```python
from build123d import *


with BuildPart() as part:
    # Sweep1: sweep along a path in Sketch1
    with BuildLine(Plane.XY) as sweep1_path:
        Line((0, 8), (1060, 8))
        ThreePointArc((1060, 8), (1068, 0), (1060, -8))
        Line((1060, -8), (0, -8))
        ThreePointArc((0, -8), (-8, 0), (0, 8))
    # Sketch2 → Sweep1 (sweep)
    with BuildSketch(Plane(origin=(0, 0, 0), x_dir=(0, 0, -1), z_dir=(1, 0, 0))):
        with BuildLine():
            Line((-10, 8), (10, 8))
            ThreePointArc((10, 8), (0, 18), (-10, 8))
        make_face()
    sweep(path=sweep1_path.line)


solid = part.part
```
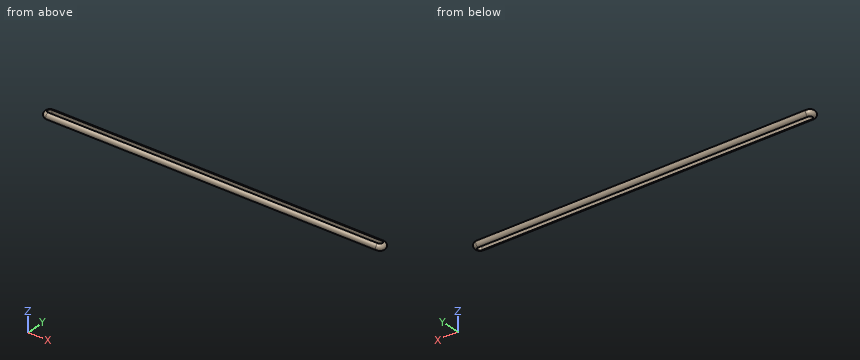
Verification items for the finished model (mm, model axes). Coordinates: 2 decimals unless noted, no trailing zeros. Write each loop counter-clockwise with the first axis right and the second up, starting at its lowest first coordinate (ties: lowest second). Pieces come first, ordered by that corner, then holes. Notation, with made-up numbers: (18.25, 76) - (68.25, 76) arc R8 ccw to (68.25, 82) - close; hole circle Ø10 at (45.5, 45.5). An arc over 180 degrees is marked (long way). One line per question, with ' | ' between items. Start each with the question number.
1. Section check A-A (x = 734). Enter the section's corners in (y, z).
2. Gauge pin test, flat ends, axial feed: P1, Ø4, axis at x = 254, y = -5.5, coming from the +Z side; P2, Ø3, axis at x = 107, y = -11, coming from the -Z side; P3, Ø4, axis at x = 477, z = -3.5, coming from the +Y side. Record the tip position at first contact, or that the pin passes through.
3. Material ranges on line 1 along Y through (x, z) = (796, 0.5); line 2 along Y through (x, z) = (788, -1.25); line 3 along X through (y, z) = (-0.5, -6), recorded low to high.
Computed values:
1) outline: (-8, -10) - (-8, 10) arc R10 ccw to start; (8, -10) arc R10 ccw to (8, 10) - close
2) P1: through | P2: z = -9.89 | P3: y = 17.89
3) line 1: -17.99 to -8, 8 to 17.99 | line 2: -17.92 to -8, 8 to 17.92 | line 3: -15.99 to -7.98, 1067.98 to 1075.99
